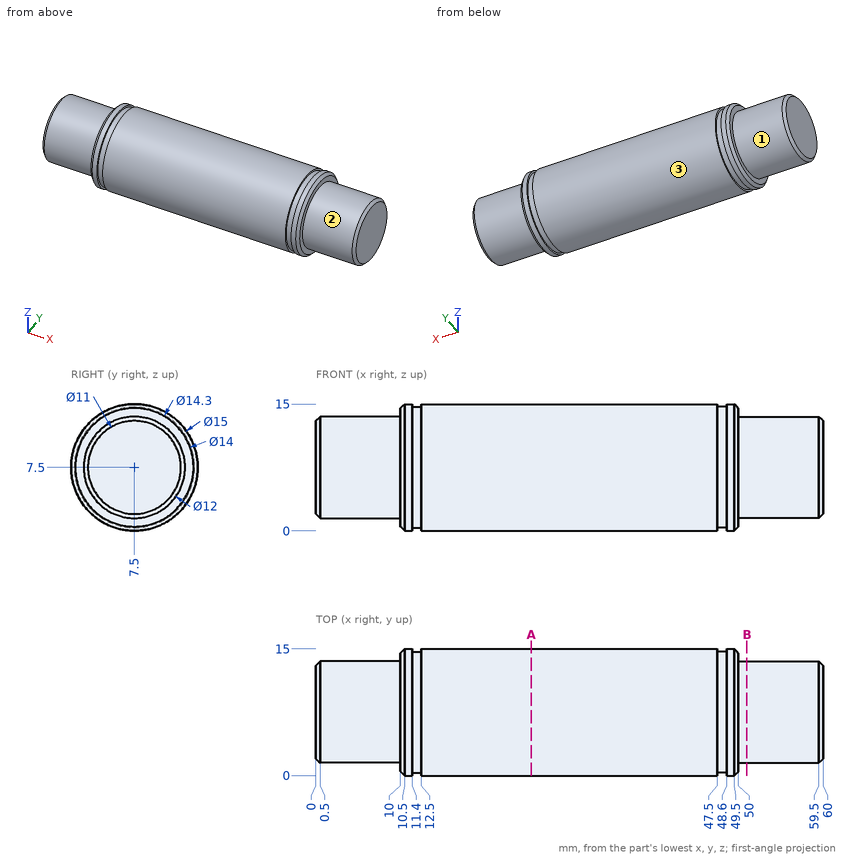
Can you work these out from the drawing? Everything is in mm from the part's minimum corner. A direction names the side the tool comes from. Give positions to 0.01 mm unless a question says otherwise; leave off trailing zeros. Order: outer loops, then holes, each group sorted by start corner. A loop starts at its lowest first (then second) coordinate and runs counter-clockwise, first axis right, second up. Notation, with made-up numbers: M 62,34 L 88,34 A20 cw 88,45 Z; hole C -13,-29.75 d3. An arc over 180 degrees is marked long. Use a Markdown table: item, result. Add a question column.
Item 1: Suppose I cut it at A-A (x = 25.5). List the corners of the cut face in (y, z) for me, then the cut area to 3 significant figures.
Item 2: Will these pins go through, and if not, where does the flat tip stop? pin 1 (1 mm diameter, centred on x = 52.5, y = 8, fed in from -Z); pin 2 (3 mm diameter, centred on y = 12, z = 2.5, fed in from -X); pin 3 (1.5 mm diameter, centred on y = 13, z = 4, fed in from +X); pin 4 (1.5 mm diameter, centred on x = 52.5, y = 5, fed in from -Z).
Item 3: Suppose I cut it at B-B (x = 51). List the corners of the cut face in (y, z) for me, then the cut area to 3 significant figures.
Item 4: If I drill on L1, parallel to X at y = 12, z = 13.25; L2, parallel to X at y = 13.5, z = 11.75; L3, parallel to Y at x = 23, z = 13, over which ranges is the centre line in solid material (lowest first)? Write a range as [from, to].
Item 5: For the marked faces 1, 2 and 3, which set-ups out of +Z, -Z, +X, -X, +Y, -Y let a thin tool reach every point of the face, with its end or its side?
Answer sheet:
| question | item | result |
|---|---|---|
| 1 | outline | C 7.5,7.5 d15 |
| 1 | area | 177 mm² |
| 2 | pin 1 | stops at z = 1.5 |
| 2 | pin 2 | stops at x = 0 |
| 2 | pin 3 | stops at x = 59.73 |
| 2 | pin 4 | stops at z = 1.76 |
| 3 | outline | C 7.5,7.5 d12 |
| 3 | area | 113 mm² |
| 4 | L1 | x = [10.3, 11.4], [12.5, 47.5], [48.6, 49.7] |
| 4 | L2 | x = [10.35, 11.4], [12.5, 47.5], [48.6, 49.65] |
| 4 | L3 | y = [2.4, 12.6] |
| 5 | face 1 | -X |
| 5 | face 2 | +X |
| 5 | face 3 | +X, -X |
